from build123d import *

# Parameters (mm, degrees)
BASE_FLANGE_SKETCH_R                 = 5
BASE_FLANGE_SKETCH_R_2               = 6
BASE_FLANGE_DEPTH                    = 10
PILLAR_AND_LUG_BOSSES_SKETCH_R       = 20
PILLAR_AND_LUG_BOSSES_SKETCH_R_2     = 5
PILLAR_AND_LUG_BOSSES_SKETCH_R_3     = 10
PILLAR_AND_LUG_BOSSES_SKETCH_R_4     = 6
PILLAR_AND_LUG_BOSSES_DEPTH          = 20
UPPER_PILLAR_SKETCH_R                = 20
UPPER_PILLAR_SKETCH_R_2              = 5
UPPER_PILLAR_40_DEPTH                = 30
SUPPORT_WEB_DEPTH                    = 5
TAPERED_BORE_SKETCH_R                = 10
TAPERED_BORE_20_DEPTH                = 15
TAPERED_BORE_20_DRAFT                = -15
TOP_FLANGE_SKETCH_R                  = 40
TOP_FLANGE_SKETCH_R_2                = 10
TOP_FLANGE_SKETCH_R_3                = 6
TOP_FLANGE_80_WITH_HOLES_4X_12_DEPTH = 16


with BuildPart() as part:
    # Base Flange Sketch → Base Flange (new body)
    with BuildSketch(Plane(origin=(0, 0, 0), x_dir=(1, 0, 0), z_dir=(0, 1, 0))):
        with BuildLine():
            Line((-11.666666667, 32.998316455), (-65, 14.142135624))
            ThreePointArc((-65, 14.142135624), (-75, 0), (-65, -14.142135624))
            Line((-65, -14.142135624), (-11.666666667, -32.998316455))
            ThreePointArc((-11.666666667, -32.998316455), (0, -35), (11.666666667, -32.998316455))
            Line((11.666666667, -32.998316455), (65, -14.142135624))
            ThreePointArc((65, -14.142135624), (75, 0), (65, 14.142135624))
            Line((65, 14.142135624), (11.666666667, 32.998316455))
            ThreePointArc((11.666666667, 32.998316455), (0, 35), (-11.666666667, 32.998316455))
        make_face()
        with Locations(Location((0, 0, 0), (0, 0, 270))):
            Circle(BASE_FLANGE_SKETCH_R, mode=Mode.SUBTRACT)
        with Locations(Location((-60, 0, 0), (0, 0, 270))):
            Circle(BASE_FLANGE_SKETCH_R_2, mode=Mode.SUBTRACT)
        with Locations(Location((60, 0, 0), (0, 0, 270))):
            Circle(BASE_FLANGE_SKETCH_R_2, mode=Mode.SUBTRACT)
    extrude(amount=BASE_FLANGE_DEPTH)

    # Pillar and Lug Bosses Sketch → Pillar and Lug Bosses (add)
    # profile 1 of 3: a face of its own
    with BuildSketch(Plane(origin=(0, 10, 0), x_dir=(1, 0, 0), z_dir=(0, 1, 0))):
        with Locations(Location((0, 0, 0), (0, 0, 270))):
            Circle(PILLAR_AND_LUG_BOSSES_SKETCH_R)
        with Locations(Location((0, 0, 0), (0, 0, 270))):
            Circle(PILLAR_AND_LUG_BOSSES_SKETCH_R_2, mode=Mode.SUBTRACT)
    # profile 2 of 3: a face of its own
    with BuildSketch(Plane(origin=(0, 10, 0), x_dir=(1, 0, 0), z_dir=(0, 1, 0))):
        with Locations(Location((-60, 0, 0), (0, 0, 270))):
            Circle(PILLAR_AND_LUG_BOSSES_SKETCH_R_3)
        with Locations(Location((-60, 0, 0), (0, 0, 270))):
            Circle(PILLAR_AND_LUG_BOSSES_SKETCH_R_4, mode=Mode.SUBTRACT)
    # profile 3 of 3: a face of its own
    with BuildSketch(Plane(origin=(0, 10, 0), x_dir=(1, 0, 0), z_dir=(0, 1, 0))):
        with Locations(Location((60, 0, 0), (0, 0, 270))):
            Circle(PILLAR_AND_LUG_BOSSES_SKETCH_R_3)
        with Locations(Location((60, 0, 0), (0, 0, 270))):
            Circle(PILLAR_AND_LUG_BOSSES_SKETCH_R_4, mode=Mode.SUBTRACT)
    extrude(amount=PILLAR_AND_LUG_BOSSES_DEPTH)

    # Upper Pillar Sketch → Upper Pillar Ø40 (add)
    with BuildSketch(Plane(origin=(0, 30, 0), x_dir=(1, 0, 0), z_dir=(0, 1, 0))):
        with Locations(Location((0, 0, 0), (0, 0, 270))):
            Circle(UPPER_PILLAR_SKETCH_R)
        with Locations(Location((0, 0, 0), (0, 0, 270))):
            Circle(UPPER_PILLAR_SKETCH_R_2, mode=Mode.SUBTRACT)
    extrude(amount=UPPER_PILLAR_40_DEPTH)

    # Support Web Sketch → Support Web (add, symmetric)
    with BuildSketch(Plane.XY):
        Polygon((-47, 30), (-52, 30), (-52, 10), (-16.568658107, 10), (-16.568658107, 60), (-20, 60), align=None)
        Polygon((52.090777917, 30), (47.090777917, 30), (20, 60), (17.352207011, 60), (17.352207011, 10), (52.090777917, 10), align=None)
    extrude(amount=SUPPORT_WEB_DEPTH, both=True)


with BuildPart() as tapered_bore_20_tool:
    # Tapered Bore Sketch → Tapered Bore Ø20 (with draft: the straight prism first)
    with BuildSketch(Plane(origin=(0, 60, 0), x_dir=(1, 0, 0), z_dir=(0, 1, 0))):
        Circle(TAPERED_BORE_SKETCH_R)
    extrude(amount=-TAPERED_BORE_20_DEPTH)
    # Tapered Bore Ø20: the draft: its side faces are tilted about the plane it starts from
    tapered_bore_20_sides = [tapered_bore_20_tool.faces().sort_by_distance(p)[0] for p in [
        (-10, 52.5, 0),
    ]]
    draft(tapered_bore_20_sides, Plane(origin=(0, 60, 0), x_dir=(1, 0, 0), z_dir=(0, 1, 0)), TAPERED_BORE_20_DRAFT)


with BuildPart() as part_1:
    add(part.part)

    # Tapered Bore Ø20: cut by tapered_bore_20_tool
    add(tapered_bore_20_tool.part, mode=Mode.SUBTRACT)

    # Top Flange Sketch → Top Flange Ø80 with Holes 4xØ12 (add)
    with BuildSketch(Plane(origin=(0, 60, 0), x_dir=(1, 0, 0), z_dir=(0, 1, 0))):
        with Locations(Location((0, 0, 0), (0, 0, 270))):
            Circle(TOP_FLANGE_SKETCH_R)
        with Locations(Location((0, 0, 0), (0, 0, 270))):
            Circle(TOP_FLANGE_SKETCH_R_2, mode=Mode.SUBTRACT)
        with Locations(Location((21.213203436, 21.213203436, 0), (0, 0, 270))):
            Circle(TOP_FLANGE_SKETCH_R_3, mode=Mode.SUBTRACT)
        with Locations(Location((21.213203436, -21.213203436, 0), (0, 0, 270))):
            Circle(TOP_FLANGE_SKETCH_R_3, mode=Mode.SUBTRACT)
        with Locations(Location((-21.213203436, -21.213203436, 0), (0, 0, 270))):
            Circle(TOP_FLANGE_SKETCH_R_3, mode=Mode.SUBTRACT)
        with Locations(Location((-21.213203436, 21.213203436, 0), (0, 0, 270))):
            Circle(TOP_FLANGE_SKETCH_R_3, mode=Mode.SUBTRACT)
    extrude(amount=TOP_FLANGE_80_WITH_HOLES_4X_12_DEPTH)


solid = part_1.part
Read the model definition and answer for the solid it produces. Units are mm, in the model's axes. A direction names the side the tool comes from. Round coordinates to 2 decimals unless told otherwise and drop trailing zeros. Order: outer loops, then holes, each group sorted by start corner. A loop starts at its lowest first (then second) coordinate and runs counter-clockwise, first axis right, second up.
1) The part is cut by section C-C on z = -30. Write down the section's boundary in (x, y), plus the area to 3 significant figures.
2) Flat-ended cylindrical pins translate along their axes: pin 1 (22 mm diameter, centred on x = 63.5, z = 4, fed in from +Y); pin 2 (15.5 mm diameter, centred on x = -21.21, z = -21.21, fed in from +Y); pin 3 (11 mm diameter, centred on x = 21.21, z = -21.21, fed in from +Y); pin 4 (12 mm diameter, centred on x = -32, y = 62, fed in from -Z). Find the tip coordinate at first contact, or state that the pin passes through.
3) Straight lines are drawn through the part: L1, parallel to X at y = 18, z = 0; L2, parallel to Y at x = -13.5, z = 16; L3, parallel to Z at x = 27.5, y = 19.5. For each, find the intervals that lie inside material, in ascending order.
4) The part is cut by section B-B on x = -60. Write down the section's boundary in (y, z).
5) For faces 1 (the face through (70, 20, 0)), 2 (the face through (53.6, 30, -0.1)), 3 (the face through (-18, 10, 15)), 4 (the face through (32, 30, -5)), 5 (the face through (-53, 30, 0)), determine the directions among +Z, -Z, +X, -X, +Y, -Y from which every point of the face is accessible in a straight line to the end or side of a thin tool.
6) The part is cut by section D-D on y = 43. Write down the section's boundary in (x, z), plus the area to 3 significant figures.
7) The part is cut by section A-A on z = 0. Give the number of separate pieces and of enclosed holes in the cut face, plus the area to 3 significant figures.
8) The mould has two halves that part along Z. Classify faces 6 (the face through (-58.198, 14.79, 5.723)), 7 (the face through (0, 35, 20)), 8 (the face through (-32, 30, -5)), 9 (the face through (-17.158, 67.888, -25.635)): released by +Z, released by -Z, zero draft, split by the parting line, or undercut.
Resolved:
1. outline: (-26.46, 60) - (26.46, 60) - (26.46, 76) - (-26.46, 76) - close; (-20.15, 0) - (20.15, 0) - (20.15, 10) - (-20.15, 10) - close
1. area: 1,250 mm2
2. pin 1: stops at y = 30
2. pin 2: stops at y = 76
2. pin 3: stops at y = 10
2. pin 4: stops at z = -30.4
3. L1: x = -70 to -66, -54 to -5, 5 to 54, 66 to 70
3. L2: y = 0 to 10, 60 to 76
3. L3: z = -5 to 5
4. outline: (0, -15.91) - (10, -15.91) - (10, -10) - (30, -10) - (30, -6) - (0, -6) - close; (0, 6) - (30, 6) - (30, 10) - (10, 10) - (10, 15.91) - (0, 15.91) - close
5. face 1: +Y
5. face 2: +Z, -Z, +X, +Y
5. face 3: none
5. face 4: -Z
5. face 5: +Z, -Z, -X, +Y
6. outline: (-35.3, -5) - (-19.36, -5) arc R20 ccw to (19.36, -5) - (35.35, -5) - (35.35, 5) - (19.36, 5) arc R20 ccw to (-19.36, 5) - (-35.3, 5) - close; hole circle Ø10 at (0, 0)
6. area: 1,490 mm2
7. separate pieces: 4
7. enclosed holes: 0
7. area: 5,860 mm2
8. face 6: undercut
8. face 7: released by +Z
8. face 8: released by -Z
8. face 9: undercut
